Verification items for the finished model (mm, model axes). Face numbers are marked on the shaded views. Give positions to 0.01 mm unless a question says otherwise; leave off trailing zeros. Write each loop counter-clockwise with the first axis right and the second up, starting at its lowest first coordinate (ties: lowest second). Pieces come first, ordered by that corner, then holes. Notation, with made-up numbers: (24.5, -34) -> (60.5, -34) arc R19 ccw to (60.5, -8) -> close; hole circle Ø10 at (44.5, 38). An arc over 180 degrees is marked (long way). Answer as CSV lines item,"result".
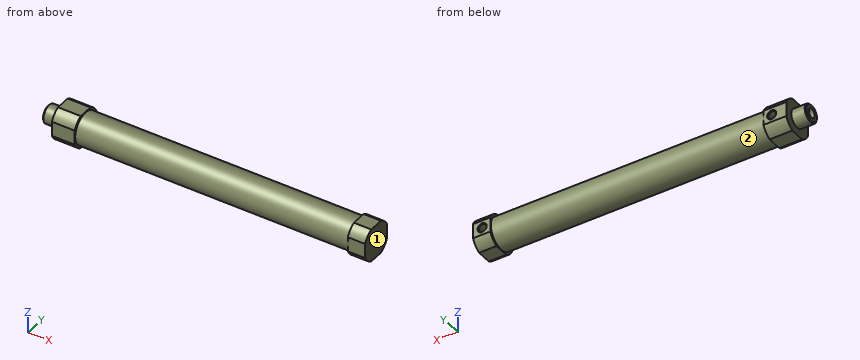
```python
from build123d import *

# Parameters (mm, degrees)
BOSS_EXTRUDE1_DEPTH = 12.5
SKETCH3_R           = 8.7
BOSS_EXTRUDE2_DEPTH = 150
BOSS_EXTRUDE3_DEPTH = 9.5
HOLE1_D             = 4.134
HOLE1_DEPTH         = 5
HOLE1_CSINK_D       = 5
HOLE1_CSINK_ANGLE   = 90
HOLE1_TIP           = 1.193383006
HOLE2_D             = 4.134
HOLE2_DEPTH         = 5
HOLE2_CSINK_D       = 5
HOLE2_CSINK_ANGLE   = 90
HOLE2_TIP           = 1.193383006


with BuildPart() as part:
    # Sketch1 → Revolve1 (revolve)
    with BuildSketch(Plane.XY, mode=Mode.PRIVATE) as revolve1_sk:
        Polygon((-8, 0), (-8, 4.3865), (-7.3865, 5), (0, 5), (0, 0), align=None)
    revolve(revolve1_sk.sketch.rotate(Axis((0, 0, 0), (-1, 0, 0)), 270), axis=Axis((0, 0, 0), (-1, 0, 0)))

    # Sketch2 → Boss-Extrude1 (add)
    with BuildSketch(Plane(origin=(0, 0, 0), x_dir=(0, 0, -1), z_dir=(1, 0, 0))):
        with BuildLine():
            Line((-4.034538387, -9.15), (4.034538387, -9.15))
            ThreePointArc((4.034538387, -9.15), (7.071067812, -7.071067812), (9.15, -4.034538387))
            Line((9.15, -4.034538387), (9.15, 4.034538387))
            ThreePointArc((9.15, 4.034538387), (7.071067812, 7.071067812), (4.034538387, 9.15))
            Line((4.034538387, 9.15), (-4.034538387, 9.15))
            ThreePointArc((-4.034538387, 9.15), (-7.071067812, 7.071067812), (-9.15, 4.034538387))
            Line((-9.15, 4.034538387), (-9.15, -4.034538387))
            ThreePointArc((-9.15, -4.034538387), (-7.071067812, -7.071067812), (-4.034538387, -9.15))
        make_face()
    extrude(amount=BOSS_EXTRUDE1_DEPTH)

    # Sketch3 → Boss-Extrude2 (add)
    with BuildSketch(Plane(origin=(12.5, 0, 0), x_dir=(0, 0, -1), z_dir=(1, 0, 0))):
        Circle(SKETCH3_R)
    extrude(amount=BOSS_EXTRUDE2_DEPTH)

    # Sketch4 → Boss-Extrude3 (add)
    with BuildSketch(Plane(origin=(162.5, 0, 0), x_dir=(0, 0, -1), z_dir=(1, 0, 0))):
        with BuildLine():
            Line((-4.034538387, -9.15), (4.034538387, -9.15))
            ThreePointArc((4.034538387, -9.15), (7.071067812, -7.071067812), (9.15, -4.034538387))
            Line((9.15, -4.034538387), (9.15, 4.034538387))
            ThreePointArc((9.15, 4.034538387), (7.071067812, 7.071067812), (4.034538387, 9.15))
            Line((4.034538387, 9.15), (-4.034538387, 9.15))
            ThreePointArc((-4.034538387, 9.15), (-7.071067812, 7.071067812), (-9.15, 4.034538387))
            Line((-9.15, 4.034538387), (-9.15, -4.034538387))
            ThreePointArc((-9.15, -4.034538387), (-7.071067812, -7.071067812), (-4.034538387, -9.15))
        make_face()
    extrude(amount=BOSS_EXTRUDE3_DEPTH)

    # Hole1
    with Locations(Plane(origin=(0, 9.15, 0), x_dir=(1, 0, 0), z_dir=(0, 1, 0))):
        with Locations((8, 0)):
            CounterSinkHole(HOLE1_D / 2, HOLE1_CSINK_D / 2, depth=HOLE1_DEPTH, counter_sink_angle=HOLE1_CSINK_ANGLE)
            with Locations((0, 0, -(HOLE1_DEPTH + HOLE1_TIP / 2))):  # 120° drill point
                Cone(0, HOLE1_D / 2, HOLE1_TIP, mode=Mode.SUBTRACT)

    # Hole2
    with Locations(Plane(origin=(0, 9.15, 0), x_dir=(1, 0, 0), z_dir=(0, 1, 0))):
        with Locations((167, 0)):
            CounterSinkHole(HOLE2_D / 2, HOLE2_CSINK_D / 2, depth=HOLE2_DEPTH, counter_sink_angle=HOLE2_CSINK_ANGLE)
            with Locations((0, 0, -(HOLE2_DEPTH + HOLE2_TIP / 2))):  # 120° drill point
                Cone(0, HOLE2_D / 2, HOLE2_TIP, mode=Mode.SUBTRACT)

    # Sketch9 → Cut-Revolve1 (revolve, cut)
    with BuildSketch(Plane.XY, mode=Mode.PRIVATE) as cut_revolve1_sk:
        Polygon((-8, 0), (-8, 2.5), (12.5, 2.5), (12.5, 8), (142.5, 8), (142.5, 0), align=None)
    revolve(cut_revolve1_sk.sketch.rotate(Axis((50, 0, 0), (-1, 0, 0)), 270), axis=Axis((50, 0, 0), (-1, 0, 0)), mode=Mode.SUBTRACT)


solid = part.part
```
1) Section check B-B (x = 69). Record the boundary of the cut face in (y, z).
Reported:
outline,"circle Ø17.4 at (0, 0); hole circle Ø16 at (0, 0)"
2) Section check C-C (y = -6.5). Record the boundary of the cut face in (x, z).
Reported:
outline,"(0, -7.6) -> (12.5, -7.6) -> (12.5, -5.78) -> (162.5, -5.78) -> (162.5, -7.6) -> (172, -7.6) -> (172, 7.6) -> (162.5, 7.6) -> (162.5, 5.78) -> (12.5, 5.78) -> (12.5, 7.6) -> (0, 7.6) -> close; hole (12.5, -4.66) -> (142.5, -4.66) -> (142.5, 4.66) -> (12.5, 4.66) -> close"
3) Depth check by flat-ended pin: pin 1 (3 mm diameter, centred on x = 107.5, z = 3, fed in from +Y); pin 2 (5 mm diameter, centred on x = 88, z = 0.5, fed in from -Y); pin 3 (5 mm diameter, centred on x = 137, z = -0.5, fed in from +Y); pin 4 (9 mm diameter, centred on y = -4.5, z = 0.5, fed in from -X). Enter the tip coordinate at first touch or a pass-through.
Reported:
pin 1,"y = 8.57"
pin 2,"y = -8.7"
pin 3,"y = 8.7"
pin 4,"x = -8"
4) Draft check along X on the marked faces 1 and 2. Enter one of: +X half, -X half, draft (parallel to the pull), parting line (faces both ways), or undercut.
Reported:
face 1,"+X half"
face 2,"undercut"
5) Scan lines: line 1 along X through (y, z) = (-6.5, 0); line 2 along X through (y, z) = (8, -1); line 3 along Y through (x, z) = (112.5, 0). Record each from-to range of solid material in increasing order.
Reported:
line 1,"0 to 12.5, 142.5 to 172"
line 2,"0 to 6.19, 9.81 to 165.19, 168.81 to 172"
line 3,"-8.7 to -8, 8 to 8.7"
6) Section check A-A (y = 0). Record the boundary of the cut face in (x, z), and give its area (3 significant figures).
Reported:
outline,"(-8, -4.39) -> (-7.39, -5) -> (0, -5) -> (0, -9.15) -> (12.5, -9.15) -> (12.5, -8.7) -> (162.5, -8.7) -> (162.5, -9.15) -> (172, -9.15) -> (172, 9.15) -> (162.5, 9.15) -> (162.5, 8.7) -> (12.5, 8.7) -> (12.5, 9.15) -> (0, 9.15) -> (0, 5) -> (-7.39, 5) -> (-8, 4.39) -> (-8, 2.5) -> (12.5, 2.5) -> (12.5, 8) -> (142.5, 8) -> (142.5, -8) -> (12.5, -8) -> (12.5, -2.5) -> (-8, -2.5) -> close"
area,"910 mm²"
